Geometry check sheet. Reference: the model listing, model coordinates, mm. A direction names the side the tool comes from. Round coordinates to 2 decimals unless told otherwise and drop trailing zeros. Order: outer loops, then holes, each group sorted by start corner. A loop starts at its lowest first (then second) coordinate and runs counter-clockwise, first axis right, second up.
(1) Cross-section at D-D on x = 48.5. Enter the section's corners in (y, z), and give its area (3 significant figures).
(2) Cross-section at B-B on x = 67.2. Enter the section's corners in (y, z), and give its area (3 significant figures).
(3) Gauge pin test, flat ends, axial feed: P1, Ø13, axis at y = -19.1, z = -11, coming from the +X side; P2, Ø12, axis at x = 35, y = -20.5, coming from the -Z side; P3, Ø9, axis at y = -19.1, z = 43, coming from the -X side. Record the tip position at first contact, or that the pin passes through.
(4) Draft check along Y on faces 1 (the face through (-7.19, -22.479, 46.685)), 2 (the face through (43, -10, -1)), 3 (the face through (-7.19, -23.316, 8.312)), 4 (the face through (26, -9, 52.5)). Enter one of: pulls with the +Y half, pulls with the -Y half, needs draft (parallel to the pull), parting line crosses it, or undercut.
(5) Cross-section at C-C on y = -19.1. Count the separate pieces of the cut face and the enclosed holes in it, and give its area (3 significant figures).
(6) Cross-section at A-A on z = -17.5. Enter the section's corners in (x, y), and give its area (3 significant figures).
(7) Thickness scan on L1, parallel to X at y = -8.5, z = -17.5; L2, parallel to Z at x = -3, y = -19; L3, parallel to Z at x = -8.05, y = -19.1. Record the ranges inside material, lowest first.
(8) Set-up check for faces 5 (the face through (-4.3, -17, 41)), 6 (the face through (88.5, -5.07, -51.07)), 7 (the face through (-2, -22, -1)): record each of +Z, -Z, +X, -X, +Y, -Y from which the full face is reachable in a straight line by a thin tool's end or side.
from build123d import *

# Parameters (mm, degrees)
EXTRUDE_1_DEPTH              = 27
SKETCH_2_R                   = 16
CUT_EXTRUDE_1_DEPTH          = 107.437775249
EXTRUDE_START                = -1.2
SKETCH_3_R                   = 16
SKETCH_3_R_2                 = 15
EXTRUDE_1_2_DEPTH            = 1.2
SKETCH_5_W                   = 100
SKETCH_5_H                   = 105
EXTRUDE_2_DEPTH              = 10
FILLET_1_R                   = 5
HOLE_WIZARD_M4_1_D           = 3.3
SKETCH_10_W                  = 21.869488537
SKETCH_10_H                  = 58.553791887
CUT_EXTRUDE_2_DEPTH          = 50
SKETCH_11_W                  = 105
SKETCH_11_H                  = 35
EXTRUDE_3_DEPTH              = 8
HOLE_WIZARD_M5_1_D           = 5.5
HOLE_WIZARD_M5_1_DEPTH       = 10.1
HOLE_WIZARD_M5_1_CBORE_D     = 10
HOLE_WIZARD_M5_1_CBORE_DEPTH = 5.7
HOLE_WIZARD_M5_1_TIP         = 1.652366702
FILLET_2_R                   = 5


with BuildPart() as part:
    # 草图1 → Extrude 1 (new, symmetric)
    with BuildSketch(Plane.XY):
        Polygon((90, 0), (0, 0), (0, 50), (-10, 50), (-10, -10), (90, -10), align=None)
    extrude(amount=EXTRUDE_1_DEPTH, both=True)

    # 草图2 → 切除-拉伸1 (cut, through all)
    with BuildSketch(Plane(origin=(0, 0, 0), x_dir=(0, 0, -1), z_dir=(1, 0, 0))):
        with Locations((0, 30)):
            Circle(SKETCH_2_R)
    extrude(amount=-CUT_EXTRUDE_1_DEPTH, mode=Mode.SUBTRACT)

    # 草图3 → Extrude 1 2 (add)
    with BuildSketch(Plane.ZY.offset(10).offset(EXTRUDE_START)):
        with Locations(Location((0, 30, 0), (0, 0, 180))):
            Circle(SKETCH_3_R)
        with Locations((0, 30)):
            Circle(SKETCH_3_R_2, mode=Mode.SUBTRACT)
    extrude(amount=EXTRUDE_1_2_DEPTH)

    # 草图5 → 凸台-拉伸2 (add)
    with BuildSketch(Plane(origin=(0, 0, 0), x_dir=(1, 0, 0), z_dir=(0, 1, 0))):
        with Locations((40, 0)):
            Rectangle(SKETCH_5_W, SKETCH_5_H)
    extrude(amount=-EXTRUDE_2_DEPTH)

    # 圆角1
    fillet_1_edges = [part.edges().sort_by_distance(p)[0] for p in [
        (-5, 50, 27),
        (90, -5, -52.5),
        (90, -5, 52.5),
        (-5, 50, -27),
    ]]
    fillet(fillet_1_edges, radius=FILLET_1_R)

    # M4 螺纹孔1 (through all)
    with Locations(Plane(origin=(67.2, 0, 17.5), x_dir=(0, 0, 1), z_dir=(0, 1, 0))):
        with Locations((0, 0), (0, -15), (-35, 0), (-35, -15)):
            Hole(HOLE_WIZARD_M4_1_D / 2)

    # 草图10 → 切除-拉伸2 (cut)
    with BuildSketch(Plane(origin=(0, 50, 0), x_dir=(1, 0, 0), z_dir=(0, 1, 0))):
        with Locations((-5.309523809, -0.493827161)):
            Rectangle(SKETCH_10_W, SKETCH_10_H)
    extrude(amount=-CUT_EXTRUDE_2_DEPTH, mode=Mode.SUBTRACT)

    # 草图11 → 凸台-拉伸3 (add)
    with BuildSketch(Plane.ZY.offset(10)):
        with Locations((0, -17.5)):
            Rectangle(SKETCH_11_W, SKETCH_11_H)
    extrude(amount=-EXTRUDE_3_DEPTH)

    # M5 六角圆柱头螺钉的柱形沉头孔1
    with Locations(Plane(origin=(-10, -19.1, -43), x_dir=(0, 0, -1), z_dir=(-1, 0, 0))):
        with Locations((0, 0), (-32, 0), (-54, 0), (-86, 0)):
            CounterBoreHole(HOLE_WIZARD_M5_1_D / 2, HOLE_WIZARD_M5_1_CBORE_D / 2, HOLE_WIZARD_M5_1_CBORE_DEPTH, depth=HOLE_WIZARD_M5_1_DEPTH)
            with Locations((0, 0, -(HOLE_WIZARD_M5_1_DEPTH + HOLE_WIZARD_M5_1_TIP / 2))):  # 118° drill point
                Cone(0, HOLE_WIZARD_M5_1_D / 2, HOLE_WIZARD_M5_1_TIP, mode=Mode.SUBTRACT)

    # 圆角2
    fillet_2_edges = [part.edges().sort_by_distance(p)[0] for p in [
        (-6, -35, -52.5),
        (-6, -35, 52.5),
    ]]
    fillet(fillet_2_edges, radius=FILLET_2_R)


solid = part.part
Found:
1. outline: (-10, -52.5) - (0, -52.5) - (0, 52.5) - (-10, 52.5) - close
1. area: 1,050 mm2
2. outline: (-10, -52.5) - (0, -52.5) - (0, -19.15) - (-10, -19.15) - close; (-10, -15.85) - (0, -15.85) - (0, 15.85) - (-10, 15.85) - close; (-10, 19.15) - (0, 19.15) - (0, 52.5) - (-10, 52.5) - close
2. area: 984 mm2
3. P1: stops at x = -2
3. P2: passes through
3. P3: stops at x = -4.3
4. face 1: undercut
4. face 2: pulls with the -Y half
4. face 3: undercut
4. face 4: needs draft
5. separate pieces: 5
5. enclosed holes: 0
5. area: 561 mm2
6. outline: (-10, -35) - (-2, -35) - (-2, -10) - (50.55, -10) - (50.55, 0) - (-10, 0) - close; (53.85, -10) - (65.55, -10) - (65.55, 0) - (53.85, 0) - close; (68.85, -10) - (90, -10) - (90, 0) - (68.85, 0) - close
6. area: 1,130 mm2
7. L1: x = -10 to 50.55, 53.85 to 65.55, 68.85 to 90
7. L2: z = -52.5 to -45.75, -40.25 to -13.75, -8.25 to 8.25, 13.75 to 40.25, 45.75 to 52.5
7. L3: z = -52.5 to -48, -38 to -16, -6 to 6, 16 to 38, 48 to 52.5
8. face 5: -X
8. face 6: -Z, +X, +Y, -Y
8. face 7: +Z, -Z, +X, -Y
